Drawing for the job (mm, zero at the part's lowest x, y, z). Coordinates: 2 decimals unless noted, no trailing zeros. Write each loop counter-clockwise with the first axis right and the second up, starting at its lowest first coordinate (ties: lowest second). Pieces come first, ordered by that corner, then holes. Notation, with made-up numbers: (-28, -33) -> (-16, -33) arc R17 ccw to (-16, -12) -> close; hole circle Ø8 at (55, 66.25). An arc over 180 degrees is marked (long way). Write each question's results on one line, items separated by ' | '. Start each with the question number.
Q1. Drill centre lines: line 1 (Y direction, x = 50, z = 11.5); line 2 (X direction, y = 62, z = 8.5); line 3 (X direction, y = 65.5, z = 9.5). Where is each one in solid material? Low to high.
Q2. Two-plate mould, pull along Y, no slides. Class the marked faces 1, 2, 3 and 4: released by +Y, released by -Y, zero draft, split by the parting line, or undercut.
Q3. Saw through at D-D on x = 11.5. Give the cut face in (y, z), and give its area (4 significant figures).
Q4. Saw through at C-C on y = 67. Give the cut face in (x, z).
Q5. Saw through at A-A on z = 3. Give the cut face in (x, y).
Q6. Drop flat-ended pins along their axis: pin 1 Ø1 at (y, z) = (65, 11.5) entering from +X; pin 2 Ø1 at (y, z) = (56.5, 10.5) entering from -X; pin 3 Ø1.5 at (x, z) = (15, 4.5) entering from +Y. Give the stop position or say it passes through.
Q7. Saw through at B-B on x = 50. Give the cut face in (y, z), and give its area (4 significant figures).
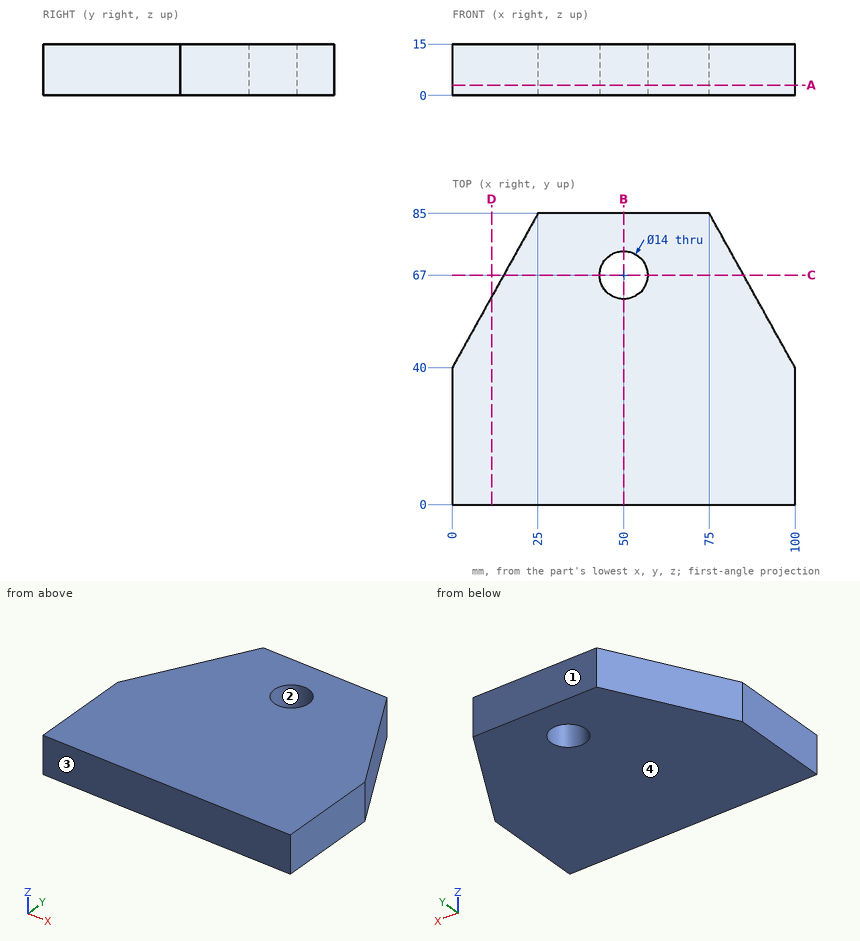
Returned:
1) line 1: y = 0 to 60, 74 to 85 | line 2: x = 12.22 to 45.1, 54.9 to 87.78 | line 3: x = 14.17 to 43.16, 56.84 to 85.83
2) face 1: released by +Y | face 2: undercut | face 3: released by -Y | face 4: zero draft
3) outline: (0, 0) -> (60.7, 0) -> (60.7, 15) -> (0, 15) -> close | area: 910.5 mm2
4) outline: (15, 0) -> (43, 0) -> (43, 15) -> (15, 15) -> close; (57, 0) -> (85, 0) -> (85, 15) -> (57, 15) -> close
5) outline: (0, 0) -> (100, 0) -> (100, 40) -> (75, 85) -> (25, 85) -> (0, 40) -> close; hole circle Ø14 at (50, 67)
6) pin 1: stops at x = 86.39 | pin 2: stops at x = 8.89 | pin 3: stops at y = 68.35
7) outline: (0, 0) -> (60, 0) -> (60, 15) -> (0, 15) -> close; (74, 0) -> (85, 0) -> (85, 15) -> (74, 15) -> close | area: 1,065 mm2
